```python
from build123d import *

# Parameters (mm, degrees)
SKETCH1_R           = 14
BOSS_EXTRUDE1_DEPTH = 3.5
SKETCH2_R           = 6
BOSS_EXTRUDE2_DEPTH = 11.5
SKETCH3_R           = 1.75
CUT_EXTRUDE1_DEPTH  = 11.5
CIRPATTERN1_COUNT   = 4
SKETCH4_R           = 3
CUT_EXTRUDE2_DEPTH  = 50


with BuildPart() as part:
    # Sketch1 → Boss-Extrude1 (new body)
    with BuildSketch(Plane.XY):
        Circle(SKETCH1_R)
    extrude(amount=BOSS_EXTRUDE1_DEPTH)

    # Sketch2 → Boss-Extrude2 (add)
    with BuildSketch(Plane.XY.offset(3.5)):
        Circle(SKETCH2_R)
    extrude(amount=BOSS_EXTRUDE2_DEPTH)

    # Sketch3 → Cut-Extrude1 (cut)
    with BuildSketch(Plane.XY.offset(3.5)):
        with Locations((0, 10)):
            Circle(SKETCH3_R)
    cut_extrude1 = extrude(amount=-CUT_EXTRUDE1_DEPTH, mode=Mode.SUBTRACT)

    # CirPattern1: Cut-Extrude1 ×4 about axis
    cirpattern1_axis = Axis((0, 0, 0), (0, 0, 1))
    for i in range(1, CIRPATTERN1_COUNT):
        add(cut_extrude1.rotate(cirpattern1_axis, i * 360 / CIRPATTERN1_COUNT), mode=Mode.SUBTRACT)

    # Sketch4 → Cut-Extrude2 (cut)
    with BuildSketch(Plane.XY.offset(15)):
        Circle(SKETCH4_R)
    extrude(amount=-CUT_EXTRUDE2_DEPTH, mode=Mode.SUBTRACT)


solid = part.part
```
For this review, take the finished solid that the model builds, in its own axes (mm). A direction names the side the tool comes from. Round coordinates to 2 decimals unless told otherwise and drop trailing zeros. Order: outer loops, then holes, each group sorted by start corner. A loop starts at its lowest first (then second) coordinate and runs counter-clockwise, first axis right, second up. Notation, with made-up numbers: (-5, 76) -> (54, 76) arc R13 cw to (54, 80) -> close; hole circle Ø6 at (55.25, 33). An arc over 180 degrees is marked (long way). Use a Markdown table: item, result.
Item 1: Take a section at A-A (x = 0). State the section outline as (y, z) points, plus the area to 4 significant figures.
Resolved:
| item | result |
|---|---|
| outline | (-14, 0) -> (-11.75, 0) -> (-11.75, 3.5) -> (-14, 3.5) -> close; (-8.25, 0) -> (-3, 0) -> (-3, 15) -> (-6, 15) -> (-6, 3.5) -> (-8.25, 3.5) -> close; (3, 0) -> (8.25, 0) -> (8.25, 3.5) -> (6, 3.5) -> (6, 15) -> (3, 15) -> close; (11.75, 0) -> (14, 0) -> (14, 3.5) -> (11.75, 3.5) -> close |
| area | 121.5 mm² |
Item 2: Take a section at C-C (x = 11.25). State the section outline as (y, z) points, plus the area to 3 significant figures.
Resolved:
| item | result |
|---|---|
| outline | (-8.33, 0) -> (-1.22, 0) -> (-1.22, 3.5) -> (-8.33, 3.5) -> close; (1.22, 0) -> (8.33, 0) -> (8.33, 3.5) -> (1.22, 3.5) -> close |
| area | 49.8 mm² |
Item 3: Draft analysis for pull direction Y (two halves, no side actions). For faces 1 (the flat face through (-3, -1, 15)), 2 (the cylindrical face through (-6, 0, 9)), 3 (the cylindrical face through (0.228, -11.735, 1.774)), state which applies: +Y half, -Y half, draft (parallel to the pull), parting line (faces both ways), or undercut.
Resolved:
| item | result |
|---|---|
| face 1 | draft |
| face 2 | parting line |
| face 3 | undercut |
Item 4: Take a section at D-D (z = 2.75). State the section outline as (x, y) points, plus the area to 3 significant figures.
Resolved:
| item | result |
|---|---|
| outline | circle Ø28 at (0, 0); hole circle Ø3.5 at (-10, 0); hole circle Ø6 at (0, 0); hole circle Ø3.5 at (0, -10); hole circle Ø3.5 at (0, 10); hole circle Ø3.5 at (10, 0) |
| area | 549 mm² |
Item 5: For line 1 along Y through (x, z) = (0, 2.5); line 2 along Z through (x, y) = (-10, -7); line 3 along Y through (x, z) = (1, 5.5), list the stretches that pass through material, from the lowest coordinate up. Write a range as [from, to].
Resolved:
| item | result |
|---|---|
| line 1 | y = [-14, -11.75], [-8.25, -3], [3, 8.25], [11.75, 14] |
| line 2 | z = [0, 3.5] |
| line 3 | y = [-5.92, -2.83], [2.83, 5.92] |
Item 6: Machinability: for faces 4 (the cylindrical face through (-0.228, 11.735, 1.774)), 5 (the flat face through (6, -3, 3.5)), which of the approach directions +Z, -Z, +X, -X, +Y, -Y give a long, thin tool a straight path to every point of the face, cutting with its end or side? Answer none if there is none.
Resolved:
| item | result |
|---|---|
| face 4 | +Z, -Z |
| face 5 | +Z |
Item 7: For pin 1 (4 mm diameter, centred on x = 10, y = 0, fed in from +Z); pin 2 (1.5 mm diameter, centred on x = 3.5, z = 2, fed in from +Y); pin 3 (4 mm diameter, centred on y = 7.5, z = 12.5, fed in from +X); pin 4 (5 mm diameter, centred on x = -10.5, z = 7, fed in from +Y) (3 decimals), all flat-tipped, find the tip position at first contact; note any pin that passes through.
Resolved:
| item | result |
|---|---|
| pin 1 | stops at z = 3.5 |
| pin 2 | stops at y = 13.73 |
| pin 3 | stops at x = 2.4 |
| pin 4 | passes through |
